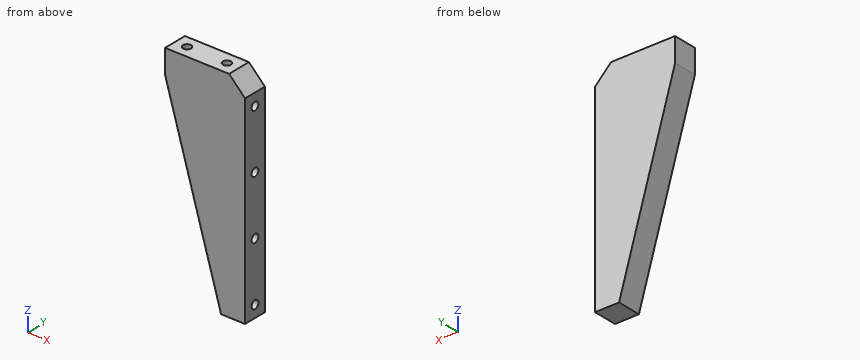
from build123d import *

# Parameters (mm, degrees)
EXTRUDE_1_DEPTH         = 30
HOLE_WIZARD_M12_1_D     = 10.2
HOLE_WIZARD_M12_1_DEPTH = 29.25
HOLE_WIZARD_M12_1_TIP   = 3.064389157
HOLE_WIZARD_M12_2_D     = 10.2
HOLE_WIZARD_M12_2_DEPTH = 29.25
HOLE_WIZARD_M12_2_TIP   = 3.064389157


with BuildPart() as part:
    # 草图1 → 凸台-拉伸1 (new body)
    with BuildSketch(Plane(origin=(0, 0, 0), x_dir=(1, 0, 0), z_dir=(0, 1, 0))):
        Polygon((0, 0), (0, -250), (-20, -270), (-100, -270), (-100, -240), (-30, 0), align=None)
    extrude(amount=EXTRUDE_1_DEPTH)

    # M12 螺纹孔1
    with Locations(Plane(origin=(0, 0, 0), x_dir=(0, 0, -1), z_dir=(1, 0, 0))):
        with Locations((-235, 15), (-15, 15), (-88.333333333, 15), (-161.666666667, 15)):
            Hole(HOLE_WIZARD_M12_1_D / 2, depth=HOLE_WIZARD_M12_1_DEPTH)
            with Locations((0, 0, -(HOLE_WIZARD_M12_1_DEPTH + HOLE_WIZARD_M12_1_TIP / 2))):  # 118° drill point
                Cone(0, HOLE_WIZARD_M12_1_D / 2, HOLE_WIZARD_M12_1_TIP, mode=Mode.SUBTRACT)

    # M12 螺纹孔2
    with Locations(Plane.XY.offset(270)):
        with Locations((-35, 15), (-85, 15)):
            Hole(HOLE_WIZARD_M12_2_D / 2, depth=HOLE_WIZARD_M12_2_DEPTH)
            with Locations((0, 0, -(HOLE_WIZARD_M12_2_DEPTH + HOLE_WIZARD_M12_2_TIP / 2))):  # 118° drill point
                Cone(0, HOLE_WIZARD_M12_2_D / 2, HOLE_WIZARD_M12_2_TIP, mode=Mode.SUBTRACT)


solid = part.part
Input: part model. Units: mm. Frame: model coordinates. Give positions to 0.01 mm unless a question says otherwise; leave off trailing zeros. Order: outer loops, then holes, each group sorted by start corner. A loop starts at its lowest first (then second) coordinate and runs counter-clockwise, first axis right, second up. Notation, with made-up numbers: (-18.5, 35) -> (13.5, 35) arc R20 ccw to (13.5, 63) -> close; hole circle Ø1 at (-23, -16.5). An arc over 180 degrees is marked (long way). Use one line per item in the form item = value.
1) First-contact query: pin 1 Ø9 at (y, z) = (15, 161.67) entering from -X; pin 2 Ø9 at (y, z) = (15, 88.33) entering from -X; pin 3 Ø4 at (x, y) = (-15.5, 25) entering from +Z. Flat tips, straight axial feed; report the tip coordinate or a pass-through.
Response values:
pin_1 = -78.47
pin_2 = -57.08
pin_3 = 267.5
2) Section C-C, the plane y = 27.25. Return loops of the section in (x, z), and give its area (3 significant figures).
Response values:
outline = (-100, 240) -> (-30, 0) -> (0, 0) -> (0, 250) -> (-20, 270) -> (-100, 270) -> close
area = 18,400 mm^2
3) Line query: probe 1 along X at (y, z) = (15, 248.75); probe 2 along Z at (x, y) = (-21.5, 15); probe 3 along X at (y, z) = (15, 255.75). Output: solid intervals per line, ascending.
Response values:
probe_1 = -100 to -90.1, -79.9 to -40.1, -29.9 to 0
probe_2 = 0 to 9.9, 20.1 to 83.23, 93.43 to 156.57, 166.77 to 229.9, 240.1 to 270
probe_3 = -100 to -90.1, -79.9 to -40.1, -29.9 to -5.75
4) Section D-D, the plane x = -58. Return loops of the section in (y, z), and give its area (3 significant figures).
Response values:
outline = (0, 96) -> (30, 96) -> (30, 270) -> (0, 270) -> close
area = 5,220 mm^2
5) Section A-A, the plane x = -26. Return loops of the section in (y, z).
Response values:
outline = (0, 0) -> (30, 0) -> (30, 270) -> (0, 270) -> close; hole circle Ø10.2 at (15, 15); hole circle Ø10.2 at (15, 88.33); hole circle Ø10.2 at (15, 161.67); hole circle Ø10.2 at (15, 235)
6) Section B-B, the plane z = 246.5. Return loops of the section in (x, y), and give its area (3 significant figures).
Response values:
outline = (-100, 0) -> (0, 0) -> (0, 30) -> (-100, 30) -> close; hole circle Ø10.2 at (-85, 15); hole circle Ø10.2 at (-35, 15)
area = 2,840 mm^2
